```python
from build123d import *

# Parameters (mm, degrees)
EXTRUDE_1_DEPTH        = 800
SKETCH_2_W             = 6
SKETCH_2_H             = 1
EXTRUDE_2_DEPTH        = 800
HOLE_WIZARD_M3_1_D     = 3.4
HOLE_WIZARD_M3_1_DEPTH = 1


with BuildPart() as part:
    # 草图1 → 拉伸-薄壁1 (new body)
    with BuildSketch(Plane.XY):
        Polygon((2.35, 5), (0, 5), (0, 0), (8, 0), (8, 5), (5.65, 5), (5.65, 4), (7, 4), (7, 1), (1, 1), (1, 4), (2.35, 4), align=None)
    extrude(amount=EXTRUDE_1_DEPTH)

    # 草图2 → 拉伸-薄壁2 (add)
    with BuildSketch(Plane.XY.offset(800)):
        with Locations((-3, 0.5)):
            Rectangle(SKETCH_2_W, SKETCH_2_H)
    extrude(amount=-EXTRUDE_2_DEPTH)

    # 镜向1: part across plane


with BuildPart() as part_1:
    add(part.part)
    add(part.part.mirror(Plane(origin=(-6, 0, -6.08276253), x_dir=(0, 0, 1), z_dir=(1, 0, 0))))

    # M3 间隙孔1
    with Locations(Plane(origin=(0, 1, 0), x_dir=(1, 0, 0), z_dir=(0, 1, 0))):
        with Locations((-16, -10), (-16, -790)):
            Hole(HOLE_WIZARD_M3_1_D / 2, depth=HOLE_WIZARD_M3_1_DEPTH)


solid = part_1.part
```
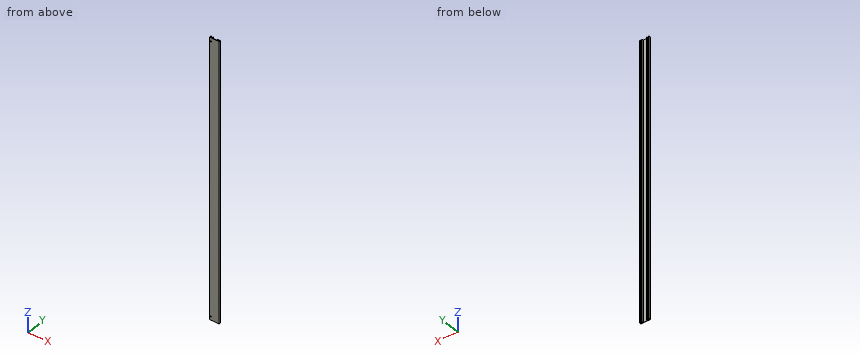
The model under review builds one solid part; all positions refer to its coordinate system, in mm. Give positions to 0.01 mm unless a question says otherwise; leave off trailing zeros. Write each loop counter-clockwise with the first axis right and the second up, starting at its lowest first coordinate (ties: lowest second). Pieces come first, ordered by that corner, then holes. Notation, with made-up numbers: (-6, 85.5) -> (38, 85.5) arc R21 cw to (38, 107.5) -> close; hole circle Ø5 at (55.25, 38). An arc over 180 degrees is marked (long way). Put each result on its own line as item: value.
(1) For pin 1 Ø1.1 at (x, z) = (-18.5, 324.5) entering from -Y; pin 2 Ø9.5 at (x, z) = (-5.5, 504) entering from +Y, all flat-tipped, find the tip position at first contact; note any pin that passes through.
Results are:
pin 1: y = 0
pin 2: y = 1
(2) We need section A-A, the plane z = 506.5. Give the boundary of the cut face in (x, y).
Results are:
outline: (-20, 0) -> (8, 0) -> (8, 5) -> (5.65, 5) -> (5.65, 4) -> (7, 4) -> (7, 1) -> (1, 1) -> (1, 4) -> (2.35, 4) -> (2.35, 5) -> (0, 5) -> (0, 1) -> (-12, 1) -> (-12, 5) -> (-14.35, 5) -> (-14.35, 4) -> (-13, 4) -> (-13, 1) -> (-19, 1) -> (-19, 4) -> (-17.65, 4) -> (-17.65, 5) -> (-20, 5) -> close
(3) To check wall thickness, follow probe 1 along X at (y, z) = (2.35, 372.5); probe 2 along X at (y, z) = (0.5, 790); probe 3 along X at (y, z) = (4.4, 220.5). State the ranges of each line that lie inside material, in increasing order. Write a range as from..to.
Results are:
probe 1: -20..-19, -13..-12, 0..1, 7..8
probe 2: -20..-17.7, -14.3..8
probe 3: -20..-17.65, -14.35..-12, 0..2.35, 5.65..8
